from build123d import *

# Parameters (mm, degrees)
SKETCH_1_R         = 20
EXTRUDE_1_DEPTH    = 4
SKETCH_2_R         = 10
EXTRUDE_2_DEPTH    = 8
SKETCH_3_R         = 7.5
EXTRUDE_3_DEPTH    = 45
SKETCH_4_W         = 0.35
SKETCH_4_H         = 1.1
HOLE_WIZARD_M5_1_D = 4.2
CHAMFER_1_SIZE     = 0.5
CHAMFER_2_SIZE     = 0.5


with BuildPart() as part:
    # 草图1 → 凸台-拉伸1 (new, symmetric)
    with BuildSketch(Plane(origin=(0, 0, 0), x_dir=(1, 0, 0), z_dir=(0, 1, 0))):
        with Locations(Location((0, 0, 0), (0, 0, 270))):
            Circle(SKETCH_1_R)
    extrude(amount=EXTRUDE_1_DEPTH, both=True)

    # 草图2 → 凸台-拉伸2 (add)
    with BuildSketch(Plane(origin=(0, 4, 0), x_dir=(1, 0, 0), z_dir=(0, 1, 0))):
        with Locations(Location((0, 0, 0), (0, 0, 270))):
            Circle(SKETCH_2_R)
    extrude(amount=EXTRUDE_2_DEPTH)

    # 草图3 → 凸台-拉伸3 (add)
    with BuildSketch(Plane(origin=(0, 12, 0), x_dir=(1, 0, 0), z_dir=(0, 1, 0))):
        with Locations(Location((0, 0, 0), (0, 0, 90))):
            Circle(SKETCH_3_R)
    extrude(amount=EXTRUDE_3_DEPTH)

    # 草图4 → 切除-旋转1 (revolve, cut)
    with BuildSketch(Plane(origin=(0, 0, 0), x_dir=(0, 0, -1), z_dir=(1, 0, 0))):
        with Locations((7.325, 53.55)):
            Rectangle(SKETCH_4_W, SKETCH_4_H)
    revolve(axis=Axis((0, 0, 0), (0, 1, 0)), mode=Mode.SUBTRACT)

    # M5 螺纹孔1 (through all)
    with Locations(Plane(origin=(0, 4, 0), x_dir=(1, 0, 0), z_dir=(0, 1, 0))):
        with Locations((-12.990381057, 7.5), (12.990381057, 7.5), (0, -15)):
            Hole(HOLE_WIZARD_M5_1_D / 2)

    # 倒角1
    chamfer_1_edges = [part.edges().sort_by_distance(p)[0] for p in [
        (0, 57, 7.5),
        (0, 12, -10),
    ]]
    chamfer(chamfer_1_edges, length=CHAMFER_1_SIZE)

    # 倒角2
    chamfer_2_edges = [part.edges().sort_by_distance(p)[0] for p in [
        (0, -4, -20),
        (0, 4, -20),
    ]]
    chamfer(chamfer_2_edges, length=CHAMFER_2_SIZE)


solid = part.part
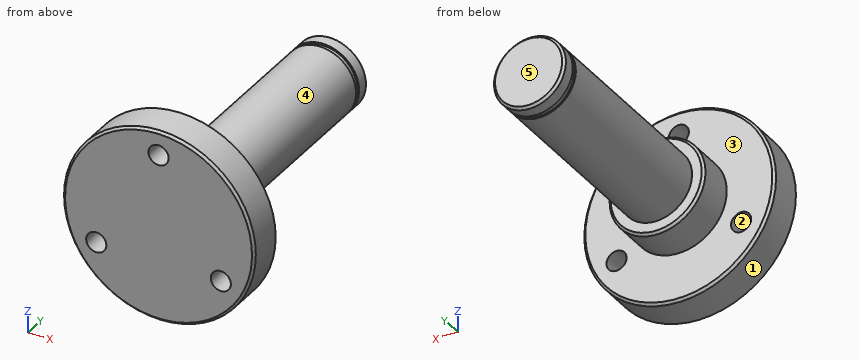
CAD build for the part. Positions are in the model's coordinates, mm. Face numbers are marked on the shaded views. A direction names the side the tool comes from. Coordinates: 2 decimals unless noted, no trailing zeros. Loops run counter-clockwise (first coordinate to the right, second up) from the corner with the lowest first, then second, coordinate; pieces in that order, holes last. Notation, with made-up numbers: (5.25, 28) -> (30.25, 28) arc R21 ccw to (30.25, 52) -> close; hole circle Ø11 at (-39.75, 37). An arc over 180 degrees is marked (long way). One line per item, written item: value.
1. Slice it at D-D on y = 9.5. Write the cut outline in (x, z), and give its area (3 significant figures).
Answers:
outline: circle Ø20 at (0, 0)
area: 314 mm^2
2. Slice it at C-C on y = 22.5. Write the cut outline in (x, z), and give its area (3 significant figures).
Answers:
outline: circle Ø15 at (0, 0)
area: 177 mm^2
3. Which spindle directions (+Z, -Z, +X, -X, +Y, -Y) get a long thin tool onto all of the face, cutting with end or side? Do the marked faces 4 and 5. Say none if no direction does.
Answers:
face 4: +Y
face 5: +Z, -Z, +X, -X, +Y
4. Drill centre lines: line 1 (Y direction, x = -14.5, z = 12); line 2 (Z direction, x = -7, y = 9); line 3 (Z direction, x = 0.5, y = 0). Where is each one in solid material? Low to high. Write a range as [from, to].
Answers:
line 1: y = [-4, 4]
line 2: z = [-7.14, 7.14]
line 3: z = [-19.99, 12.96], [17.04, 19.99]
5. Slice it at B-B on z = 0. Write the cut outline in (x, y).
Answers:
outline: (-20, -3.5) -> (-19.5, -4) -> (19.5, -4) -> (20, -3.5) -> (20, 3.5) -> (19.5, 4) -> (10, 4) -> (10, 11.5) -> (9.5, 12) -> (7.5, 12) -> (7.5, 53) -> (7.15, 53) -> (7.15, 54.1) -> (7.5, 54.1) -> (7.5, 56.5) -> (7, 57) -> (-7, 57) -> (-7.5, 56.5) -> (-7.5, 54.1) -> (-7.15, 54.1) -> (-7.15, 53) -> (-7.5, 53) -> (-7.5, 12) -> (-9.5, 12) -> (-10, 11.5) -> (-10, 4) -> (-19.5, 4) -> (-20, 3.5) -> close
6. Pull direction X, two halves, no side cores. Call the marked faces 1, 2 and 3: pulls with the +X half, pulls with the -X half, needs draft (parallel to the pull), parting line crosses it, or undercut.
Answers:
face 1: parting line crosses it
face 2: undercut
face 3: needs draft
7. Flat gauge pins, fed straight in: P1, Ø6, axis at x = -15.5, z = -1, coming from the +Y side; P2, Ø1.5, axis at x = 5, y = 48, coming from the +Z side; P3, Ø5, axis at y = 32, z = -2, coming from the -X side; P4, Ø1.5, axis at x = -15.5, z = -14.5, coming from the -Y side. Where does each tip first touch, or does it go through?
Answers:
P1: stops at y = 4
P2: stops at z = 6.18
P3: stops at x = -7.5
P4: passes through
